```python
from build123d import *

# Parameters (mm, degrees)
BOSS_EXTRUDE1_DEPTH = 66.78
SKETCH3_W           = 8.06
SKETCH3_H           = 55.56
BOSS_EXTRUDE2_DEPTH = 40
SKETCH5_W           = 71.144376366
SKETCH5_H           = 69.78
BOSS_EXTRUDE4_DEPTH = 2.5
SKETCH6_W           = 73.144376366
SKETCH6_H           = 71.78
BOSS_EXTRUDE5_DEPTH = 2.5
SKETCH7_R           = 1.5
CUT_EXTRUDE1_DEPTH  = 10


with BuildPart() as part:
    # Sketch1 → Boss-Extrude1 (new body)
    with BuildSketch(Plane.XY):
        with BuildLine():
            Line((-34.072188183, 25.498094011), (34.072188183, 25.498094011))
            Line((34.072188183, 25.498094011), (34.072188183, -16.561905989))
            Line((34.072188183, -16.561905989), (30.370310886, -18.699185843))
            ThreePointArc((30.370310886, -18.699185843), (30.140310886, -18.699185843), (30.025310886, -18.5))
            Line((30.025310886, -18.5), (30.025310886, -10.173149416))
            ThreePointArc((30.025310886, -10.173149416), (17.215197166, -1.899763481), (2.201193992, 0.77))
            Line((2.201193992, 0.77), (0, 0.77))
            Line((0, 0.77), (-2.201193992, 0.77))
            ThreePointArc((-2.201193992, 0.77), (-17.215197166, -1.899763481), (-30.025310886, -10.173149416))
            Line((-30.025310886, -10.173149416), (-30.025310886, -18.5))
            ThreePointArc((-30.025310886, -18.5), (-30.140310886, -18.699185843), (-30.370310886, -18.699185843))
            Line((-30.370310886, -18.699185843), (-34.072188183, -16.561905989))
            Line((-34.072188183, -16.561905989), (-34.072188183, 25.498094011))
        make_face()
    extrude(amount=-BOSS_EXTRUDE1_DEPTH)

    # Sketch3 → Boss-Extrude2 (add)
    with BuildSketch(Plane(origin=(0, 25.498094011, 0), x_dir=(1, 0, 0), z_dir=(0, 1, 0))):
        with Locations((0, 33.39)):
            Rectangle(SKETCH3_W, SKETCH3_H)
    extrude(amount=-BOSS_EXTRUDE2_DEPTH)

    # Sketch5 → Boss-Extrude4 (add)
    with BuildSketch(Plane(origin=(0, 25.498094011, 0), x_dir=(1, 0, 0), z_dir=(0, 1, 0))):
        with Locations((0, 33.39)):
            Rectangle(SKETCH5_W, SKETCH5_H)
    extrude(amount=BOSS_EXTRUDE4_DEPTH)

    # Sketch6 → Boss-Extrude5 (add)
    with BuildSketch(Plane(origin=(0, 27.998094011, 0), x_dir=(1, 0, 0), z_dir=(0, 1, 0))):
        with Locations((0, 33.39)):
            Rectangle(SKETCH6_W, SKETCH6_H)
    extrude(amount=BOSS_EXTRUDE5_DEPTH)

    # Sketch7 → Cut-Extrude1 (cut)
    with BuildSketch(Plane(origin=(0, 0, -66.78), x_dir=(-1, 0, 0), z_dir=(0, 0, -1))):
        with Locations((0, 6.101165809)):
            Circle(SKETCH7_R)
        with Locations((0, 16.101165809)):
            Circle(SKETCH7_R)
    extrude(amount=-CUT_EXTRUDE1_DEPTH, mode=Mode.SUBTRACT)


solid = part.part
```
The model under review builds one solid part; all positions refer to its coordinate system, in mm. A direction names the side the tool comes from. Round coordinates to 2 decimals unless told otherwise and drop trailing zeros. Write each loop counter-clockwise with the first axis right and the second up, starting at its lowest first coordinate (ties: lowest second). Pieces come first, ordered by that corner, then holes. Notation, with made-up numbers: M 72.5,46 L 99.5,46 A24 ccw 99.5,83 Z; hole C 19,26 d4. An arc over 180 degrees is marked long. Use CSV: the item, a comma, the result in double quotes. Start each with the question number.
(1) We need section A-A, the plane y = -12. State the section outline as (x, z) points, then the cut area to 3 significant figures.
(2) The part is to be moulded in two halves that separate along X. For faces 6 (the face through (-1, 29, -69.28)), 7 (the face through (-32.195, -17.646, -32.923)), 8 (the face through (30.025, -14, -33)), say which applies: +X half, -X half, draft (parallel to the pull), parting line (faces both ways), or undercut.
(3) For line 1 along Y through (x, z) = (0, -62.5); line 2 along Y through (x, z) = (0, -60); line 3 along X through (y, z) = (-10.5, -7), list the stretches that pass through material, from the lowest coordinate up.
(4) Clearance check with flat-ended pins moving along their axes: P1, Ø6, axis at x = 1.5, z = -48, coming from the -Y side; P2, Ø1.5, axis at x = -16.5, y = 7.5, coming from the +Z side; P3, Ø9, axis at y = -13.5, z = -41.5, coming from the -X side. State where each tip first meets the part, or that it passes through.
(5) We need section C-C, the plane z = -20. State the section outline as (x, y) points, then the cut area to 3 significant figures.
(6) Tool access review of faces 1 (the face through (0, -7, -5.61)), 2 (the face through (0, 16, -56.78)), 3 (the face through (0, 9, -66.78)), 4 (the face through (4.03, -7, -33)), 5 (the face through (0, 27, 1.5)): name each direction out of +Z, -Z, +X, -X, +Y, -Y from which nothing blocks a thin tool from reaching the whole face with its end or side.
(7) We need section D-D, the plane z = -63. State the section outline as (x, y) points.
(8) We need section B-B, the plane x = 0. State the section outline as (y, z) points.
Findings:
1,outline,"M -34.07,-66.78 L -30.03,-66.78 L -30.03,0 L -34.07,0 Z; M -4.03,-61.17 L 4.03,-61.17 L 4.03,-5.61 L -4.03,-5.61 Z; M 30.03,-66.78 L 34.07,-66.78 L 34.07,0 L 30.03,0 Z"
1,area,"988 mm^2"
2,face 6,"draft"
2,face 7,"-X half"
2,face 8,"undercut"
3,line 1,"0.77 to 4.6, 7.6 to 14.6, 17.6 to 30.5"
3,line 2,"-14.5 to 4.6, 7.6 to 14.6, 17.6 to 30.5"
3,line 3,"-34.07 to -30.03, -4.03 to 4.03, 30.03 to 34.07"
4,P1,"y = -14.5"
4,P2,"z = 0"
4,P3,"x = -34.07"
5,outline,"M -36.57,28 L -35.57,28 L -35.57,25.5 L -34.07,25.5 L -34.07,-16.56 L -30.37,-18.7 A0.23 ccw -30.03,-18.5 L -30.03,-10.17 A38.62 cw -4.03,0.77 L -4.03,-14.5 L 4.03,-14.5 L 4.03,0.77 A38.62 cw 30.03,-10.17 L 30.03,-18.5 A0.23 ccw 30.37,-18.7 L 34.07,-16.56 L 34.07,25.5 L 35.57,25.5 L 35.57,28 L 36.57,28 L 36.57,30.5 L -36.57,30.5 Z"
5,area,"2,500 mm^2"
6,face 1,"+Z, -Y"
6,face 2,"-Z"
6,face 3,"-Z, +X, -X, -Y"
6,face 4,"+Z, -Z, -Y"
6,face 5,"+Z, +X, -X, -Y"
7,outline,"M -36.57,28 L -35.57,28 L -35.57,25.5 L -34.07,25.5 L -34.07,-16.56 L -30.37,-18.7 A0.23 ccw -30.03,-18.5 L -30.03,-10.17 A38.62 cw -2.2,0.77 L 2.2,0.77 A38.62 cw 30.03,-10.17 L 30.03,-18.5 A0.23 ccw 30.37,-18.7 L 34.07,-16.56 L 34.07,25.5 L 35.57,25.5 L 35.57,28 L 36.57,28 L 36.57,30.5 L -36.57,30.5 Z; hole C 0,6.1 d3; hole C 0,16.1 d3"
8,outline,"M -14.5,-61.17 L 0.77,-61.17 L 0.77,-66.78 L 4.6,-66.78 L 4.6,-56.78 L 7.6,-56.78 L 7.6,-66.78 L 14.6,-66.78 L 14.6,-56.78 L 17.6,-56.78 L 17.6,-66.78 L 25.5,-66.78 L 25.5,-68.28 L 28,-68.28 L 28,-69.28 L 30.5,-69.28 L 30.5,2.5 L 28,2.5 L 28,1.5 L 25.5,1.5 L 25.5,0 L 0.77,0 L 0.77,-5.61 L -14.5,-5.61 Z"
